Work out the finished part from the listing and answer in its coordinate system (mm). Coordinates: 2 decimals unless noted, no trailing zeros. Order: outer loops, then holes, each group sorted by start corner. A loop starts at its lowest first (then second) coordinate and runs counter-clockwise, first axis right, second up.
1. Flat-ended cylindrical pins translate along their axes: pin 1 Ø1.5 at (x, z) = (17.5, 78.5) entering from +Y; pin 2 Ø2 at (y, z) = (-9.5, 126.5) entering from +X; pin 3 Ø12 at (x, y) = (10, -19) entering from -Z. Find the tip coordinate at first contact, or state that the pin passes through.
2. Find the intervals of material crossed by probe 1 along Z at (x, y) = (10.5, -3); probe 2 along Y at (x, z) = (20.5, 140.5); probe 3 along Y at (x, z) = (-3.5, 180.5), in increasing order.
3. The part is cut by section D-D, the plane x = 20. Give the vertices of the cut face in (y, z), then the cut area to 3 significant figures.
4. The part is cut by section A-A, the plane x = 0. Give the vertices of the cut face in (y, z).
5. The part is cut by section C-C, the plane z = 163.5. Give the vertices of the cut face in (x, y).
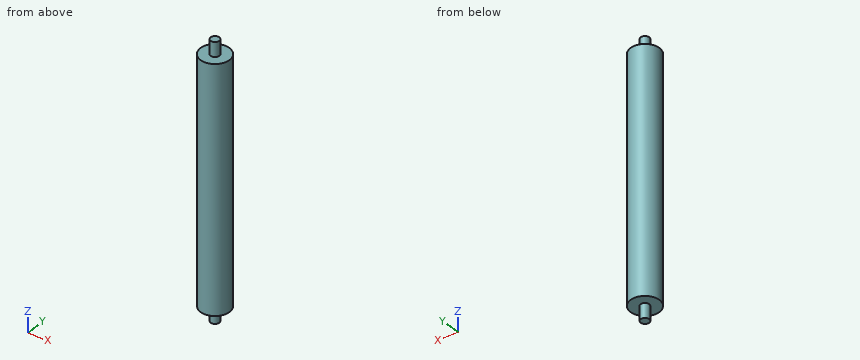
```python
from build123d import *

# Parameters (mm, degrees)
SKETCH_1_R      = 25
EXTRUDE_1_DEPTH = 420
SKETCH_2_R      = 7.5
EXTRUDE_2_DEPTH = 25
EXTRUDE_START   = 25
SKETCH_3_R      = 7.5
EXTRUDE_3_DEPTH = 25


with BuildPart() as part:
    # 草图1 → 凸台-拉伸1 (new body)
    with BuildSketch(Plane.XY):
        Circle(SKETCH_1_R)
    extrude(amount=EXTRUDE_1_DEPTH)

    # 草图2 → 凸台-拉伸2 (add)
    with BuildSketch(Plane.XY.offset(420)):
        Circle(SKETCH_2_R)
    extrude(amount=EXTRUDE_2_DEPTH)

    # 草图3 → 凸台-拉伸3 (add)
    with BuildSketch(Plane(origin=(0, 0, 0), x_dir=(-1, 0, 0), z_dir=(0, 0, -1)).offset(EXTRUDE_START)):
        with Locations(Location((0, 0, 0), (0, 0, 180))):
            Circle(SKETCH_3_R)
    extrude(amount=-EXTRUDE_3_DEPTH)


solid = part.part
```
Geometry says:
1. pin 1: stops at y = 18.56
1. pin 2: stops at x = 23.51
1. pin 3: stops at z = 0
2. probe 1: z = 0 to 420
2. probe 2: y = -14.31 to 14.31
2. probe 3: y = -24.75 to 24.75
3. outline: (-15, 0) - (15, 0) - (15, 420) - (-15, 420) - close
3. area: 12,600 mm2
4. outline: (-25, 0) - (-7.5, 0) - (-7.5, -25) - (7.5, -25) - (7.5, 0) - (25, 0) - (25, 420) - (7.5, 420) - (7.5, 445) - (-7.5, 445) - (-7.5, 420) - (-25, 420) - close
5. outline: circle Ø50 at (0, 0)
